```python
from build123d import *

# Parameters (mm, degrees)
SKETCH_1_W                = 100
SKETCH_1_H                = 71.5
EXTRUDE_1_DEPTH           = 8
CUT_EXTRUDE_1_DEPTH       = 10
FILLET_1_R                = 10
CHAMFER_2_SIZE            = 2
SKETCH_4_R                = 17.5
CUT_EXTRUDE_2_DEPTH       = 5
HOLE_WIZARD_1_D           = 4.5
HOLE_WIZARD_1_CBORE_D     = 7.5
HOLE_WIZARD_1_CBORE_DEPTH = 4.5


with BuildPart() as part:
    # 草图1 → 凸台-拉伸1 (new body)
    with BuildSketch(Plane.XY):
        Rectangle(SKETCH_1_W, SKETCH_1_H)
    extrude(amount=EXTRUDE_1_DEPTH)

    # 草图3 → 切除-拉伸1 (cut)
    with BuildSketch(Plane(origin=(0, 0, 0), x_dir=(-1, 0, 0), z_dir=(0, 0, -1))):
        Polygon((-50, 10.25), (-40, 35.75), (-50, 35.75), align=None)
        Polygon((50, 35.75), (50, 10.25), (40, 35.75), align=None)
    extrude(amount=-CUT_EXTRUDE_1_DEPTH, mode=Mode.SUBTRACT)

    # 圆角1
    fillet_1_edges = [part.edges().sort_by_distance(p)[0] for p in [
        (50, 10.25, 4),
        (40, 35.75, 4),
        (-40, 35.75, 4),
        (-50, 10.25, 4),
    ]]
    fillet(fillet_1_edges, radius=FILLET_1_R)

    # 倒角2
    chamfer_2_edges = [part.edges().sort_by_distance(p)[0] for p in [
        (50, -35.75, 4),
        (-50, -35.75, 4),
    ]]
    chamfer(chamfer_2_edges, length=CHAMFER_2_SIZE)

    # 草图4 → 切除-拉伸2 (cut)
    with BuildSketch(Plane(origin=(0, 0, 0), x_dir=(-1, 0, 0), z_dir=(0, 0, -1))):
        with Locations((0, 8.75)):
            Circle(SKETCH_4_R)
    extrude(amount=-CUT_EXTRUDE_2_DEPTH, mode=Mode.SUBTRACT)

    # 打孔尺寸(%根据)内六角圆柱头螺钉的类型1 (through all)
    with Locations(Plane.XY.offset(8)):
        with Locations((-45, 5.25), (-43.15, -26.75), (45, 5.25), (43.15, -26.75)):
            CounterBoreHole(HOLE_WIZARD_1_D / 2, HOLE_WIZARD_1_CBORE_D / 2, HOLE_WIZARD_1_CBORE_DEPTH)


solid = part.part
```
Geometry check sheet. Reference: the model listing, model coordinates, mm. A direction names the side the tool comes from. Give positions to 0.01 mm unless a question says otherwise; leave off trailing zeros. Write each loop counter-clockwise with the first axis right and the second up, starting at its lowest first coordinate (ties: lowest second). Pieces come first, ordered by that corner, then holes. Notation, with made-up numbers: (37.25, 85) - (94.25, 85) arc R23 ccw to (94.25, 107) - close; hole circle Ø1 at (-17.5, 89.25). An arc over 180 degrees is marked (long way). Use a Markdown table: item, result.
Q1. Thickness scan on L1, parallel to X at y = 4.5, z = 5.5; L2, parallel to Y at x = 0, z = 4.75; L3, parallel to Z at x = -10, y = 10. Record the ranges inside material, lowest first. Write a range as [from, to].
Computed:
| item | result |
|---|---|
| L1 | x = [-50, -48.67], [-41.33, 41.33], [48.67, 50] |
| L2 | y = [-35.75, -8.75], [26.25, 35.75] |
| L3 | z = [5, 8] |
Q2. Section check A-A, the plane y = -26.75. Enter the section's corners in (x, z), then the cut area to 3 significant figures.
Computed:
| item | result |
|---|---|
| outline | (-50, 0) - (-45.4, 0) - (-45.4, 3.5) - (-46.9, 3.5) - (-46.9, 8) - (-50, 8) - close; (-40.9, 0) - (40.9, 0) - (40.9, 3.5) - (39.4, 3.5) - (39.4, 8) - (-39.4, 8) - (-39.4, 3.5) - (-40.9, 3.5) - close; (45.4, 0) - (50, 0) - (50, 8) - (46.9, 8) - (46.9, 3.5) - (45.4, 3.5) - close |
| area | 701 mm² |
Q3. Section check C-C, the plane x = 10. Enter the section's corners in (y, z).
Computed:
| item | result |
|---|---|
| outline | (-35.75, 0) - (-5.61, 0) - (-5.61, 5) - (23.11, 5) - (23.11, 0) - (35.75, 0) - (35.75, 8) - (-35.75, 8) - close |
Q4. Section check D-D, the plane y = 5.25. Enter the section's corners in (x, z), then the cut area to 3 significant figures.
Computed:
| item | result |
|---|---|
| outline | (-50, 0) - (-47.25, 0) - (-47.25, 3.5) - (-48.75, 3.5) - (-48.75, 8) - (-50, 8) - close; (-42.75, 0) - (-17.15, 0) - (-17.15, 5) - (17.15, 5) - (17.15, 0) - (42.75, 0) - (42.75, 3.5) - (41.25, 3.5) - (41.25, 8) - (-41.25, 8) - (-41.25, 3.5) - (-42.75, 3.5) - close; (47.25, 0) - (50, 0) - (50, 8) - (48.75, 8) - (48.75, 3.5) - (47.25, 3.5) - close |
| area | 530 mm² |
Q5. Go/stop test with flat-tipped pins: P1, Ø4, axis at x = -43.15, y = -26.75, coming from the +Z side; P2, Ø1.5, axis at y = 25, z = 1, coming from the +X side; P3, Ø7, axis at x = -43.15, y = -26.75, coming from the +Z side; P4, Ø3, axis at y = 26, z = 6, coming from the -X side. Record where each tip stops, or that it passes through.
Computed:
| item | result |
|---|---|
| P1 | passes through |
| P2 | stops at x = 44.51 |
| P3 | stops at z = 3.5 |
| P4 | stops at x = -44.41 |
Q6. Draft check along X on faces 4 (the face through (41.254, 5.415, 5.781)), 5 (the face through (0, 35.75, 4)), 6 (the face through (49.01, -34.74, 3.94)). Enter one of: pulls with the +X half, pulls with the -X half, needs draft (parallel to the pull), parting line crosses it, or undercut.
Computed:
| item | result |
|---|---|
| face 4 | undercut |
| face 5 | needs draft |
| face 6 | pulls with the +X half |
Q7. Section check B-B, the plane z = 2.5. Enter the section's corners in (x, y), then the cut area to 3 significant figures.
Computed:
| item | result |
|---|---|
| outline | (-50, -33.75) - (-48, -35.75) - (48, -35.75) - (50, -33.75) - (50, 8.36) arc R10 ccw to (49.31, 12.01) - (42.49, 29.4) arc R10 ccw to (33.18, 35.75) - (-33.18, 35.75) arc R10 ccw to (-42.49, 29.4) - (-49.31, 12.01) arc R10 ccw to (-50, 8.36) - close; hole circle Ø4.5 at (-45, 5.25); hole circle Ø4.5 at (-43.15, -26.75); hole circle Ø35 at (0, 8.75); hole circle Ø4.5 at (43.15, -26.75); hole circle Ø4.5 at (45, 5.25) |
| area | 5,850 mm² |
Q8. Set-up check for faces 1 (the face through (49.82, 10.24, 4.06)), 2 (the face through (46.614, -28.186, 5.781)), 3 (the face through (13.887, -1.898, 2.465)): record each of +Z, -Z, +X, -X, +Y, -Y from which the full face is reachable in a straight line by a thin tool's end or side.
Computed:
| item | result |
|---|---|
| face 1 | +Z, -Z, +X, +Y |
| face 2 | +Z |
| face 3 | -Z |
